```python
from build123d import *

# Parameters (mm, degrees)
SKETCH_1_R          = 13
SKETCH_1_R_2        = 8.5
EXTRUDE_1_DEPTH     = 18
SKETCH_2_R          = 23.5
EXTRUDE_2_DEPTH     = 20
SKETCH_3_R          = 8.5
CUT_EXTRUDE_1_DEPTH = 39.787884706
SKETCH_4_R          = 5
EXTRUDE_3_DEPTH     = 6
CHAMFER_1_SIZE      = 0.5


with BuildPart() as part:
    # 草图1 → 拉伸1 (new body)
    with BuildSketch(Plane(origin=(0, 0, 0), x_dir=(1, 0, 0), z_dir=(0, 1, 0))):
        with Locations(Location((0, 0, 0), (0, 0, 270))):
            Circle(SKETCH_1_R)
        with Locations(Location((0, 0, 0), (0, 0, 270))):
            Circle(SKETCH_1_R_2, mode=Mode.SUBTRACT)
    extrude(amount=EXTRUDE_1_DEPTH)

    # 草图2 → 拉伸2 (add)
    with BuildSketch(Plane(origin=(0, 18, 0), x_dir=(-1, 0, 0), z_dir=(0, 1, 0))):
        with Locations(Location((0, 0, 0), (0, 0, 90))):
            Circle(SKETCH_2_R)
    extrude(amount=EXTRUDE_2_DEPTH)

    # 草图3 → 切除-拉伸1 (cut, through all)
    with BuildSketch(Plane.XZ.offset(-18)):
        with Locations(Location((0, 0, 0), (0, 0, 270))):
            Circle(SKETCH_3_R)
    extrude(amount=-CUT_EXTRUDE_1_DEPTH, mode=Mode.SUBTRACT)

    # 草图4 → 拉伸3 (add)
    with BuildSketch(Plane(origin=(0, 38, 0), x_dir=(-1, 0, 0), z_dir=(0, 1, 0))):
        with Locations(Location((-18.25, 0, 0), (0, 0, 90))):
            Circle(SKETCH_4_R)
        with Locations(Location((-9.125, 15.804963619, 0), (0, 0, 90))):
            Circle(SKETCH_4_R)
        with Locations(Location((9.125, 15.804963619, 0), (0, 0, 90))):
            Circle(SKETCH_4_R)
        with Locations(Location((18.25, 0, 0), (0, 0, 90))):
            Circle(SKETCH_4_R)
        with Locations(Location((9.125, -15.804963619, 0), (0, 0, 90))):
            Circle(SKETCH_4_R)
        with Locations(Location((-9.125, -15.804963619, 0), (0, 0, 90))):
            Circle(SKETCH_4_R)
    extrude(amount=EXTRUDE_3_DEPTH)

    # 倒角1
    chamfer_1_edges = [part.edges().sort_by_distance(p)[0] for p in [
        (0, 0, -13),
        (0, 0, -8.5),
        (0, 18, -23.5),
    ]]
    chamfer(chamfer_1_edges, length=CHAMFER_1_SIZE)


solid = part.part
```
For this review, take the finished solid that the model builds, in its own axes (mm). A direction names the side the tool comes from. Coordinates: 2 decimals unless noted, no trailing zeros. Order: outer loops, then holes, each group sorted by start corner. A loop starts at its lowest first (then second) coordinate and runs counter-clockwise, first axis right, second up. Notation, with made-up numbers: (-11, -10.75) - (20, -10.75) arc R21 ccw to (20, 17.25) - close; hole circle Ø3 at (12, 5). An arc over 180 degrees is marked (long way). Answer as a JSON object with one key per item and string values. Group by question number.
1. We need section A-A on z = 0. State the section outline as (x, y) points.
2. For faces 4 (the cylindrical face through (-23.13, 40.96, -1.08)), 5 (the flat face through (-10, 18, 10)), 6 (the flat face through (9, 44, -16)), list the 3-axis set-ups (+Z, -Z, +X, -X, +Y, -Y) from which the entire face can be reached by the end or side of a thin tool; tool diameter is ignored.
3. We need section B-B on x = 0. State the section outline as (y, z) points.
4. We need section C-C on y = 10. State the section outline as (x, z) points.
5. We need section D-D on y = 25. State the section outline as (x, z) points.
6. For probe 1 along X at (y, z) = (22.75, 0); probe 2 along X at (y, z) = (11.75, 0); probe 3 along Y at (x, z) = (-6.5, 7.5), list the stretches that pass through material, from the lowest coordinate up.
7. Clearance check with flat-ended pins moving along their axes: P1, Ø12, axis at y = 39.5, z = -10.5, coming from the +X side; P2, Ø8, axis at y = 7.5, z = 2, coming from the +X side; P3, Ø1, axis at x = -2, y = 7, coming from the +Z side; P4, Ø13.5, axis at x = 0, z = 0, coming from the -Y side. State where each tip first meets the part, or that it passes through.
8. The part is to be moulded in two halves that separate along Z. For faces 1 (the cylindrical face through (13.37, 40.96, -1.08)), 2 (the flat face through (3, 0, -9)), 3 (the cylindrical face through (-7.91, 9.128, -10.316)), say which applies: pulls with the +Z half, pulls with the -Z half, needs draft (parallel to the pull), parting line crosses it, or undercut.
Final values:
{
 "1": {"outline": "(-23.5, 18.5) - (-23, 18) - (-13, 18) - (-13, 0.5) - (-12.5, 0) - (-9, 0) - (-8.5, 0.5) - (-8.5, 38) - (-13.25, 38) - (-13.25, 44) - (-23.25, 44) - (-23.25, 38) - (-23.5, 38) - close; (8.5, 0.5) - (9, 0) - (12.5, 0) - (13, 0.5) - (13, 18) - (23, 18) - (23.5, 18.5) - (23.5, 38) - (23.25, 38) - (23.25, 44) - (13.25, 44) - (13.25, 38) - (8.5, 38) - close"},
 "2": {"face 4": "+Y", "face 5": "-Y", "face 6": "+Z, -Z, +X, -X, +Y"},
 "3": {"outline": "(0, -12.5) - (0.5, -13) - (18, -13) - (18, -23) - (18.5, -23.5) - (38, -23.5) - (38, -8.5) - (0.5, -8.5) - (0, -9) - close; (0, 9) - (0.5, 8.5) - (38, 8.5) - (38, 23.5) - (18.5, 23.5) - (18, 23) - (18, 13) - (0.5, 13) - (0, 12.5) - close"},
 "4": {"outline": "circle Ø26 at (0, 0); hole circle Ø17 at (0, 0)"},
 "5": {"outline": "circle Ø47 at (0, 0); hole circle Ø17 at (0, 0)"},
 "6": {"probe 1": "-23.5 to -8.5, 8.5 to 23.5", "probe 2": "-13 to -8.5, 8.5 to 13", "probe 3": "0 to 38"},
 "7": {"P1": "x = 23.03", "P2": "x = 13", "P3": "z = 12.91", "P4": "through"},
 "8": {"face 1": "undercut", "face 2": "needs draft", "face 3": "parting line crosses it"}
}
